Geometry check sheet. Reference: the model listing, model coordinates, mm. Give positions to 0.01 mm unless a question says otherwise; leave off trailing zeros. Order: outer loops, then holes, each group sorted by start corner. A loop starts at its lowest first (then second) coordinate and runs counter-clockwise, first axis right, second up.
from build123d import *

# Parameters (mm, degrees)
HEX_BODY_DEPTH                        = 2.5
BORE_SKETCH_R                         = 2
BORE_4_DEPTH                          = 15.142135624
CORNER_CHAMFER_SKETCH_OUTSIDE_W       = 37.386
CORNER_CHAMFER_SKETCH_OUTSIDE_H       = 34.706
CORNER_CHAMFER_SKETCH_OUTSIDE_R       = 8.660254038
CORNER_CHAMFER_45DEG_DEPTH            = 5
CORNER_CHAMFER_45DEG_DRAFT            = -45
CORNER_CHAMFER_MIRROR_COPY_1_SKETCH_W = 37.386
CORNER_CHAMFER_MIRROR_COPY_1_SKETCH_H = 34.706
CORNER_CHAMFER_MIRROR_COPY_1_SKETCH_R = 8.660254038
CORNER_CHAMFER_MIRROR_COPY_1_DEPTH    = 5
CORNER_CHAMFER_MIRROR_COPY_1_DRAFT    = -45


with BuildPart() as part:
    # Hex Profile Sketch → Hex Body (new, symmetric)
    with BuildSketch(Plane.XY):
        Polygon((10, 0), (5, 8.660254038), (-5, 8.660254038), (-10, 0), (-5, -8.660254038), (5, -8.660254038), align=None)
    extrude(amount=HEX_BODY_DEPTH, both=True)

    # Bore Sketch → Bore Ø4 (cut, through all)
    with BuildSketch(Plane.XY.offset(2.5)):
        Circle(BORE_SKETCH_R)
    extrude(amount=-BORE_4_DEPTH, mode=Mode.SUBTRACT)


with BuildPart() as corner_chamfer_45deg_tool:
    # Corner Chamfer Sketch outside → Corner Chamfer 45deg (with draft: the straight prism first)
    with BuildSketch(Plane.XY.offset(2.5)):
        Rectangle(CORNER_CHAMFER_SKETCH_OUTSIDE_W, CORNER_CHAMFER_SKETCH_OUTSIDE_H)
        Circle(CORNER_CHAMFER_SKETCH_OUTSIDE_R, mode=Mode.SUBTRACT)
    extrude(amount=-CORNER_CHAMFER_45DEG_DEPTH)
    # Corner Chamfer 45deg: the draft: its side faces are tilted about the plane it starts from
    corner_chamfer_45deg_sides = [corner_chamfer_45deg_tool.faces().sort_by_distance(p)[0] for p in [
        (0, -17.353, 0),
        (18.693, 0, 0),
        (0, 17.353, 0),
        (-18.693, 0, 0),
        (-8.660254038, 0, 0),
    ]]
    draft(corner_chamfer_45deg_sides, Plane.XY.offset(2.5), CORNER_CHAMFER_45DEG_DRAFT)


with BuildPart() as part_1:
    add(part.part)

    # Corner Chamfer 45deg: cut by corner_chamfer_45deg_tool
    add(corner_chamfer_45deg_tool.part, mode=Mode.SUBTRACT)


with BuildPart() as corner_chamfer_mirror_copy_1_tool:
    # Corner Chamfer Mirror copy 1 sketch → Corner Chamfer Mirror copy 1 (with draft: the straight prism first)
    with BuildSketch(Plane(origin=(0, 0, -2.5), x_dir=(1, 0, 0), z_dir=(0, 0, -1))):
        Rectangle(CORNER_CHAMFER_MIRROR_COPY_1_SKETCH_W, CORNER_CHAMFER_MIRROR_COPY_1_SKETCH_H)
        Circle(CORNER_CHAMFER_MIRROR_COPY_1_SKETCH_R, mode=Mode.SUBTRACT)
    extrude(amount=-CORNER_CHAMFER_MIRROR_COPY_1_DEPTH)
    # Corner Chamfer Mirror copy 1: the draft: its side faces are tilted about the plane it starts from
    corner_chamfer_mirror_copy_1_sides = [corner_chamfer_mirror_copy_1_tool.faces().sort_by_distance(p)[0] for p in [
        (0, -17.353, 0),
        (18.693, 0, 0),
        (0, 17.353, 0),
        (-18.693, 0, 0),
        (-8.660254038, 0, 0),
    ]]
    draft(corner_chamfer_mirror_copy_1_sides, Plane(origin=(0, 0, -2.5), x_dir=(1, 0, 0), z_dir=(0, 0, -1)), CORNER_CHAMFER_MIRROR_COPY_1_DRAFT)


with BuildPart() as part_2:
    add(part_1.part)

    # Corner Chamfer Mirror copy 1: cut by corner_chamfer_mirror_copy_1_tool
    add(corner_chamfer_mirror_copy_1_tool.part, mode=Mode.SUBTRACT)


solid = part_2.part
Item 1: Gauge pin test, flat ends, axial feed: pin 1 (6.5 mm diameter, centred on x = 0, y = 0, fed in from +Z); pin 2 (1.5 mm diameter, centred on y = -4.5, z = 0.5, fed in from -X); pin 3 (3 mm diameter, centred on y = -2.5, z = 1.5, fed in from -X). Record the tip position at first contact, or that the pin passes through.
Reported:
pin 1: stops at z = 2.5
pin 2: stops at x = -7.83
pin 3: stops at x = -9.42
Item 2: Scan lines: L1, parallel to Y at x = 0, z = -0.15; L2, parallel to Y at x = 1.25, z = -1.55; L3, parallel to X at y = -1.5, z = 0.55. Record each from-to range of solid material in increasing order.
Reported:
L1: y = -8.66 to -2, 2 to 8.66
L2: y = -8.66 to -1.56, 1.56 to 8.66
L3: x = -9.13 to -1.32, 1.32 to 9.13
Item 3: Draft check along X on faces 1 (the conical face through (8.98, 0.02, -2.18)), 2 (the cylindrical face through (0, -2, 0)), 3 (the flat face through (0, -8.66, 0)). Enter one of: released by +X, released by -X, zero draft, split by the parting line, or undercut.
Reported:
face 1: released by +X
face 2: undercut
face 3: zero draft
Item 4: Sectioned sample at B-B (z = -1.7). Enter the section's corners in (x, y), and give its area (3 significant figures).
Reported:
outline: (-9.4, -1.03) - (-5.6, -7.63) arc R9.46 ccw to (-3.81, -8.66) - (3.81, -8.66) arc R9.46 ccw to (5.6, -7.63) - (9.4, -1.03) arc R9.46 ccw to (9.4, 1.03) - (5.6, 7.63) arc R9.46 ccw to (3.81, 8.66) - (-3.81, 8.66) arc R9.46 ccw to (-5.6, 7.63) - (-9.4, 1.03) arc R9.46 ccw to start; hole circle Ø4 at (0, 0)
area: 244 mm2
Item 5: Sectioned sample at A-A (z = 0.55). Enter the section's corners in (x, y), and give its area (3 significant figures).
Reported:
outline: (-10, 0) - (-5, -8.66) - (5, -8.66) - (10, 0) - (5, 8.66) - (-5, 8.66) - close; hole circle Ø4 at (0, 0)
area: 247 mm2
